Work out the finished part from the listing and answer in its coordinate system (mm). Round coordinates to 2 decimals unless told otherwise and drop trailing zeros. Write each loop counter-clockwise with the first axis right and the second up, starting at its lowest first coordinate (ties: lowest second). Pieces come first, ordered by that corner, then holes.
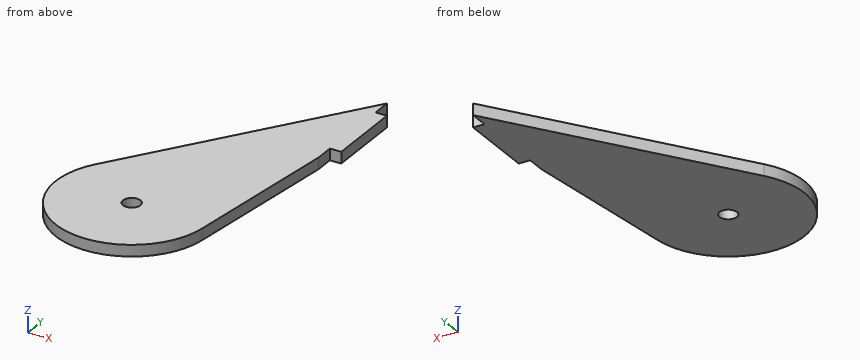
from build123d import *

# Parameters (mm, degrees)
BOSS_EXTRUDE1_DEPTH = 3
SKETCH2_R           = 2.3
CUT_EXTRUDE1_DEPTH  = 10
SKETCH4_W           = 3
SKETCH4_H           = 20
BOSS_EXTRUDE3_DEPTH = 3


with BuildPart() as part:
    # Sketch1 → Boss-Extrude1 (new body)
    with BuildSketch(Plane.XY):
        with BuildLine():
            Line((-16.33027103, 11.546525368), (25, 70))
            Line((25, 70), (25, 40))
            Line((25, 40), (19.854388756, -2.408992972))
            ThreePointArc((19.854388756, -2.408992972), (-7.196803073, -18.660279353), (-16.33027103, 11.546525368))
        make_face()
    extrude(amount=-BOSS_EXTRUDE1_DEPTH)

    # Sketch2 → Cut-Extrude1 (cut)
    with BuildSketch(Plane.XY):
        Circle(SKETCH2_R)
    extrude(amount=-CUT_EXTRUDE1_DEPTH, mode=Mode.SUBTRACT)

    # Sketch4 → Boss-Extrude3 (add)
    with BuildSketch(Plane(origin=(25, 0, 0), x_dir=(0, 0, -1), z_dir=(1, 0, 0))):
        with Locations((1.5, 55)):
            Rectangle(SKETCH4_W, SKETCH4_H)
    extrude(amount=BOSS_EXTRUDE3_DEPTH)


solid = part.part
Q1. Given pin 1 (1.5 mm diameter, centred on x = 27, z = -2, fed in from +Y); pin 2 (1.5 mm diameter, centred on x = 26.5, z = -2, fed in from -Y), each flat-ended and moving along its own axis, determine where each tip first touches the part or whether it passes through.
Q2. Find the intervals of material crossed by L1, parallel to Y at x = 0, z = -0.6; L2, parallel to X at y = 53, z = -1.1; L3, parallel to Y at x = -17.5, z = -0.8, in increasing order.
Q3. Find section B-B (x = 0). Determine the outline of the cut face in (y, z).
Q4. Find section D-D (y = 19.5). Determine the outline of the cut face in (x, z), plus the area to 3 significant figures.
Q5. Find section C-C (y = 0). Determine the outline of the cut face in (x, z).
Q6. Find section A-A (z = -1.55). Determine the outline of the cut face in (x, y), plus the area to 3 significant figures.
Report:
1. pin 1: stops at y = 65
1. pin 2: stops at y = 45
2. L1: y = -20 to -2.3, 2.3 to 34.64
2. L2: x = 12.98 to 28
2. L3: y = -9.68 to 9.68
3. outline: (-20, -3) - (-2.3, -3) - (-2.3, 0) - (-20, 0) - close; (2.3, -3) - (34.64, -3) - (34.64, 0) - (2.3, 0) - close
4. outline: (-10.71, -3) - (22.51, -3) - (22.51, 0) - (-10.71, 0) - close
4. area: 99.7 mm2
5. outline: (-20, -3) - (-2.3, -3) - (-2.3, 0) - (-20, 0) - close; (2.3, -3) - (20.15, -3) - (20.15, 0) - (2.3, 0) - close
6. outline: (-16.33, 11.55) arc R20 ccw (long way) to (19.85, -2.41) - (25, 40) - (25, 45) - (28, 45) - (28, 65) - (25, 65) - (25, 70) - close; hole circle Ø4.6 at (0, 0)
6. area: 2,290 mm2
